Here's the drawing with two shaded views (mm, measured from the low corner). I have some questions. Coordinates: 2 decimals unless noted, no trailing zeros. Loops run counter-clockwise (first coordinate to the right, second up) from the corner with the lowest first, then second, coordinate; pieces in that order, holes last. Notation, with made-up numbers: (20.5, -4.5) - (45.5, -4.5) arc R20 cw to (45.5, 14.5) - close; hole circle Ø9 at (65.25, 20). An arc over 180 degrees is marked (long way). Use a Markdown table: item, result.
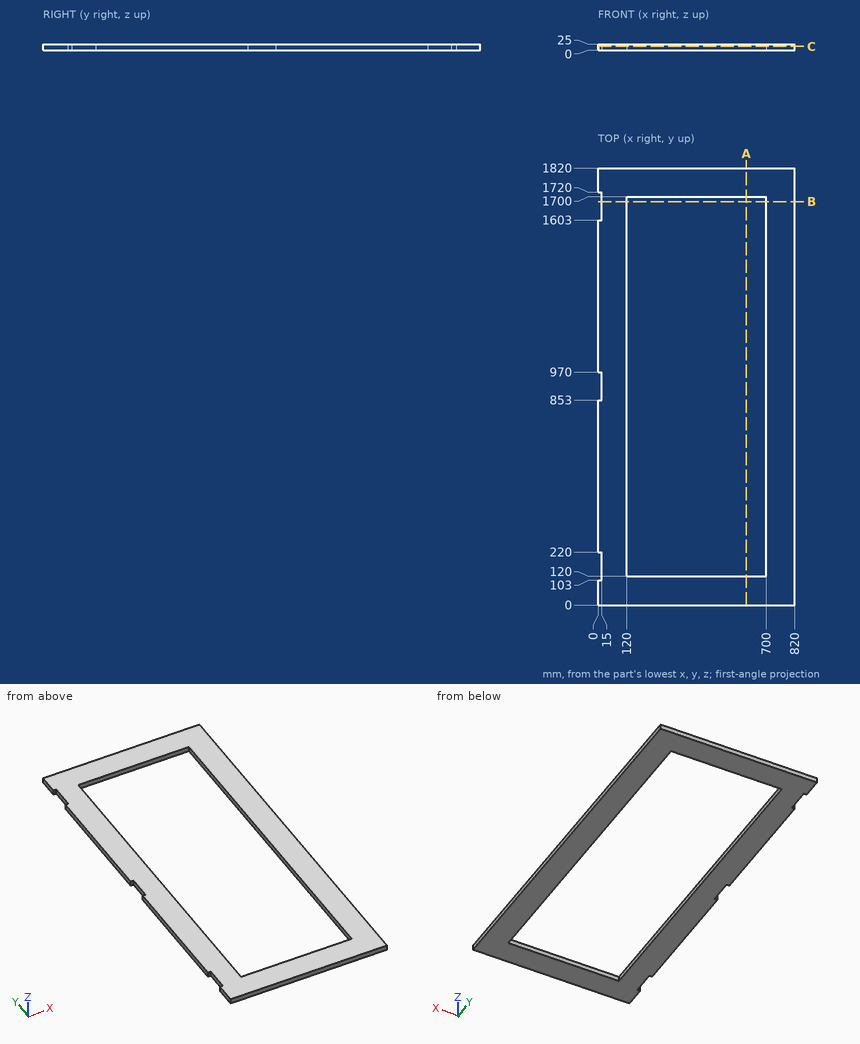
Q1. Please list where these lines run through material, in increasing order: L1, parallel to X at y = 780.5, z = 15.25; L2, parallel to Y at x = 381.5, z = 10; L3, parallel to X at y = 1613.5, z = 11.25. Write a range as from..to.
Check values:
| item | result |
|---|---|
| L1 | 0..120, 700..820 |
| L2 | 0..120, 1700..1820 |
| L3 | 15..120, 700..820 |
Q2. I want a section at C-C, the plane z = 15.25. Write out the boundary of the cut face in (x, y).
Check values:
| item | result |
|---|---|
| outline | (0, 0) - (820, 0) - (820, 1820) - (0, 1820) - (0, 1720) - (15, 1720) - (15, 1603) - (0, 1603) - (0, 970) - (15, 970) - (15, 853) - (0, 853) - (0, 220) - (15, 220) - (15, 103) - (0, 103) - close; hole (120, 120) - (700, 120) - (700, 1700) - (120, 1700) - close |
Q3. Will this pin go through, and if not, where does the flat tip stop? P1, Ø7.5, axis at y = 940.5, z = 9, coming from the -X side.
Check values:
| item | result |
|---|---|
| P1 | x = 15 |
Q4. I want a section at A-A, the plane x = 617. Write out the boundary of the cut face in (y, z).
Check values:
| item | result |
|---|---|
| outline | (0, 0) - (120, 0) - (120, 25) - (0, 25) - close; (1700, 0) - (1820, 0) - (1820, 25) - (1700, 25) - close |
Q5. I want a section at B-B, the plane y = 1680.5. Write out the boundary of the cut face in (x, z).
Check values:
| item | result |
|---|---|
| outline | (15, 0) - (120, 0) - (120, 25) - (15, 25) - close; (700, 0) - (820, 0) - (820, 25) - (700, 25) - close |
